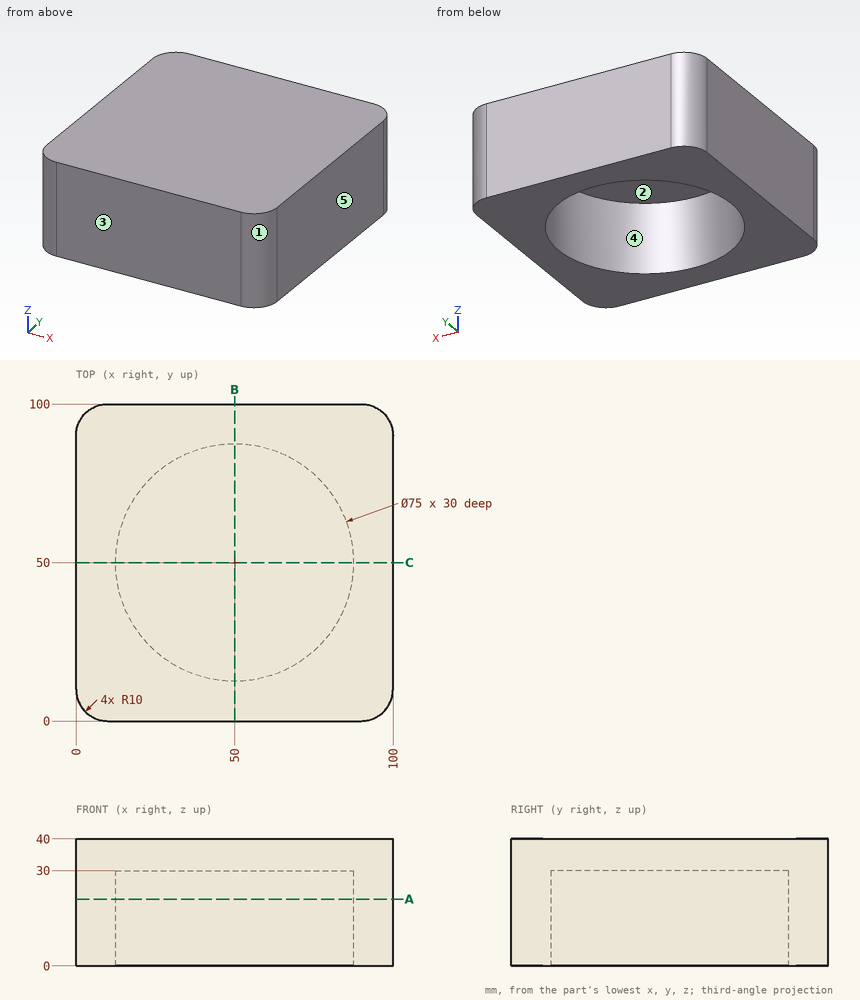
Could you check a few things on this drawing? It's one solid part, dimensions in mm from its lowest x, y, z. A direction names the side the tool comes from. Give positions to 0.01 mm unless a question says otherwise; leave off trailing zeros. Write each loop counter-clockwise with the first axis right and the second up, starting at its lowest first coordinate (ties: lowest second). Pieces come first, ordered by that corner, then holes.
(1) On a 3-axis mill with a long thin cutter (end or side, diameter ignored), from which of +Z, -Z, +X, -X, +Y, -Y can I reach the whole of each face in a straight line? I mean the marked faces 1 and 2. Say none if no direction works.
Output values:
face 1: +Z, -Z, +X, -Y
face 2: -Z
(2) Thinking about a two-plate mould opening in X: for the marked faces 3, 4 and 5, which applies, pulls with the +X half, pulls with the -X half, needs draft (parallel to the pull), parting line crosses it, or undercut?
Output values:
face 3: needs draft
face 4: undercut
face 5: pulls with the +X half
(3) If I drill on L1, parallel to Y at x = 50, z = 21.5; L2, parallel to Z at x = 25.5, y = 67.5; L3, parallel to Y at x = 18, z = 21.5, over which ranges is the centre line in solid material (lowest first)?
Output values:
L1: y = 0 to 12.5, 87.5 to 100
L2: z = 30 to 40
L3: y = 0 to 30.45, 69.55 to 100
(4) Will this pin go through, and if not, where does the flat tip stop? pin 1 (3 mm diameter, centred on x = 38.5, y = 39, fed in from -Z).
Output values:
pin 1: stops at z = 30
(5) Imagine slicing it at A-A, the plane z = 21. Write out the boundary of the cut face in (x, y), and give its area (3 significant figures).
Output values:
outline: (0, 10) arc R10 ccw to (10, 0) - (90, 0) arc R10 ccw to (100, 10) - (100, 90) arc R10 ccw to (90, 100) - (10, 100) arc R10 ccw to (0, 90) - close; hole circle Ø75 at (50, 50)
area: 5,500 mm2
(6) Imagine slicing it at B-B, the plane x = 50. Write out the boundary of the cut face in (y, z).
Output values:
outline: (0, 0) - (12.5, 0) - (12.5, 30) - (87.5, 30) - (87.5, 0) - (100, 0) - (100, 40) - (0, 40) - close
